Here's how the part is built. I have some questions about the finished solid (model axes, mm). A direction names the side the tool comes from. Coordinates: 2 decimals unless noted, no trailing zeros. Order: outer loops, then holes, each group sorted by start corner. A loop starts at its lowest first (then second) coordinate and runs counter-clockwise, first axis right, second up. Notation, with made-up numbers: (-31.75, 78) - (13.25, 78) arc R24 ccw to (13.25, 107) - close; hole circle Ø4 at (65, 9.25). An arc over 180 degrees is marked (long way). Answer as CSV lines item,"result". Start each with the question number.
Item 1: I need wall thicknesses on line 1 (Y direction, x = 75, z = 11); line 2 (X direction, y = 188.5, z = 15.25); line 3 (X direction, y = 105.5, z = 1.75). Which ranges of each line are inside material? Lowest first, please.
Item 2: Imagine slicing it at A-A on y = 30. List the corners of the cut face in (x, z) for me, and give its area (3 significant figures).
Item 3: On a 3-axis mill with a long thin cutter (end or side, diameter ignored), from which of +Z, -Z, +X, -X, +Y, -Y can I reach the whole of each face in a straight line? I mean faces 1 (the face through (150, 99, 10)), 2 (the face through (81, 20, 10)), 3 (the face through (69, 180, 10)). Say none if no direction works.
Item 4: Imagine slicing it at B-B on x = 75. List the corners of the cut face in (y, z) for me, and give its area (3 significant figures).
Item 5: We'd pull the mould along Y, two halves only. Please class faces 4 (the face through (55, 85, 10)), 5 (the face through (0, 101, 10)), 6 (the face through (35, 200, 10)): pulls with the +Y half, pulls with the -Y half, needs draft (parallel to the pull), parting line crosses it, or undercut.
Item 6: Imagine slicing it at C-C on z = 14.25. List the corners of the cut face in (x, y) for me, and give its area (3 significant figures).
from build123d import *

# Parameters (mm, degrees)
SKETCH1_R           = 25
BOSS_EXTRUDE1_DEPTH = 20


with BuildPart() as part:
    # Sketch1 → Boss-Extrude1 (new body)
    with BuildSketch(Plane.XY):
        with BuildLine():
            Line((0, 0), (69, 0))
            Line((69, 0), (69, 39))
            ThreePointArc((69, 39), (75, 45), (81, 39))
            Line((81, 39), (81, 0))
            Line((81, 0), (150, 0))
            Line((150, 0), (150, 200))
            Line((150, 200), (81, 200))
            Line((81, 200), (81, 161))
            ThreePointArc((81, 161), (75, 155), (69, 161))
            Line((69, 161), (69, 200))
            Line((69, 200), (0, 200))
            Line((0, 200), (0, 0))
        make_face()
        with Locations((75, 100)):
            Circle(SKETCH1_R, mode=Mode.SUBTRACT)
    extrude(amount=BOSS_EXTRUDE1_DEPTH)


solid = part.part
Responses:
1,line 1,"y = 45 to 75, 125 to 155"
1,line 2,"x = 0 to 69, 81 to 150"
1,line 3,"x = 0 to 50.61, 99.39 to 150"
2,outline,"(0, 0) - (69, 0) - (69, 20) - (0, 20) - close; (81, 0) - (150, 0) - (150, 20) - (81, 20) - close"
2,area,"2,760 mm^2"
3,face 1,"+Z, -Z, +X, +Y, -Y"
3,face 2,"+Z, -Z, -Y"
3,face 3,"+Z, -Z, +Y"
4,outline,"(45, 0) - (75, 0) - (75, 20) - (45, 20) - close; (125, 0) - (155, 0) - (155, 20) - (125, 20) - close"
4,area,"1,200 mm^2"
5,face 4,"undercut"
5,face 5,"needs draft"
5,face 6,"pulls with the +Y half"
6,outline,"(0, 0) - (69, 0) - (69, 39) arc R6 cw to (81, 39) - (81, 0) - (150, 0) - (150, 200) - (81, 200) - (81, 161) arc R6 cw to (69, 161) - (69, 200) - (0, 200) - close; hole circle Ø50 at (75, 100)"
6,area,"27,000 mm^2"
